```python
from build123d import *

# Parameters (mm, degrees)
SKETCH2_R          = 10.5
SKETCH2_R_2        = 8
CUT_EXTRUDE1_DEPTH = 1
CUT_EXTRUDE2_START = -1
SKETCH3_R          = 10.5
SKETCH3_R_2        = 8
CUT_EXTRUDE2_DEPTH = 1


with BuildPart() as part:
    # Sketch1 → Revolve1 (revolve)
    with BuildSketch(Plane.XY, mode=Mode.PRIVATE) as revolve1_sk:
        Polygon((0, 6), (6, 6), (6, 12), (1.5, 12), (1.5, 13.25), (0, 13.25), align=None)
    revolve(revolve1_sk.sketch.rotate(Axis((0, 0, 0), (1, 0, 0)), 90), axis=Axis((0, 0, 0), (1, 0, 0)))

    # Sketch2 → Cut-Extrude1 (cut)
    with BuildSketch(Plane(origin=(6, 0, 0), x_dir=(0, 0, -1), z_dir=(1, 0, 0))):
        Circle(SKETCH2_R)
        Circle(SKETCH2_R_2, mode=Mode.SUBTRACT)
    extrude(amount=-CUT_EXTRUDE1_DEPTH, mode=Mode.SUBTRACT)

    # Sketch3 → Cut-Extrude2 (cut)
    with BuildSketch(Plane.ZY.offset(CUT_EXTRUDE2_START)):
        with Locations(Location((0, 0, 0), (0, 0, 180))):
            Circle(SKETCH3_R)
        with Locations(Location((0, 0, 0), (0, 0, 180))):
            Circle(SKETCH3_R_2, mode=Mode.SUBTRACT)
    extrude(amount=CUT_EXTRUDE2_DEPTH, mode=Mode.SUBTRACT)


solid = part.part
```
Source: CAD feature listing. Evaluate the final solid. Frame: model axes, mm. A direction names the side the tool comes from. Round coordinates to 2 decimals unless told otherwise and drop trailing zeros. Write each loop counter-clockwise with the first axis right and the second up, starting at its lowest first coordinate (ties: lowest second). Pieces come first, ordered by that corner, then holes. Notation, with made-up numbers: M 52,-10 L 86,-10 A24 cw 86,5 Z; hole C -9,0 d5. An arc over 180 degrees is marked long. Use CSV: the item, a comma, the result in double quotes. Start each with the question number.
Q1. First-contact query: P1, Ø1, axis at x = 1, z = 1.5, coming from the +Y side; P2, Ø2, axis at x = 1, z = -9, coming from the +Y side; P3, Ø2, axis at x = 1, y = 4.5, coming from the -Z side. Flat tips, straight axial feed; report the tip coordinate or a pass-through.
Q2. Cut plane D-D on y = 11.5. Output: boundary loops of the cut face in (x, z).
Q3. Access query for faces 1 (the face through (5.51, -7.81, 1.73)), 2 (the face through (0.74, -13.137, -1.725)), 3 (the face through (0.51, 7.81, 1.73)). Directions: +Z, -Z, +X, -X, +Y, -Y. A direction counts if a zero-diameter tool reaches every point of the face in a straight line with its end or side. Return the directions, or none.
Q4. Line query: line 1 (Y direction, x = 5.3, z = 0); line 2 (Y direction, x = 1.9, z = 0); line 3 (Y direction, x = 0.55, z = -6.25). Output: solid intervals per line, ascending. Write a range as from..to.
Q5. Cut plane C-C on x = 0.5. Output: boundary loops of the cut face in (y, z), plus the area to 3 significant figures.
Q6. Cut plane A-A on z = 0. Output: boundary loops of the cut face in (x, y), plus the area to 4 significant figures.
Q7. Pull-direction query (Y, two-part tool) for faces 4 (the face through (0.5, -3.2, -10)), 5 (the face through (3.718, -3.604, 11.446)), 6 (the face through (5.5, 3.2, -10)), 7 (the face through (6, 11, 0)); classes: +Y half, -Y half, draft (parallel to the pull), parting line (faces both ways), or undercut.
Results found:
1,P1,"y = 13.21"
1,P2,"y = 10.56"
1,P3,"z = -12.78"
2,outline,"M 0,-6.58 L 1.5,-6.58 L 1.5,-3.43 L 6,-3.43 L 6,3.43 L 1.5,3.43 L 1.5,6.58 L 0,6.58 Z"
3,face 1,"+X"
3,face 2,"+X, -X"
3,face 3,"-X"
4,line 1,"-12..-10.5, -8..-6, 6..8, 10.5..12"
4,line 2,"-12..-6, 6..12"
4,line 3,"-11.68..-8.44, -4.99..4.99, 8.44..11.68"
5,outline,"C 0,0 d26.5; C 0,0 d16; hole C 0,0 d21; hole C 0,0 d12"
5,area,"293 mm^2"
6,outline,"M 0,-13.25 L 1.5,-13.25 L 1.5,-12 L 6,-12 L 6,-10.5 L 5,-10.5 L 5,-8 L 6,-8 L 6,-6 L 0,-6 L 0,-8 L 1,-8 L 1,-10.5 L 0,-10.5 Z; M 0,6 L 6,6 L 6,8 L 5,8 L 5,10.5 L 6,10.5 L 6,12 L 1.5,12 L 1.5,13.25 L 0,13.25 L 0,10.5 L 1,10.5 L 1,8 L 0,8 Z"
6,area,"65.75 mm^2"
7,face 4,"undercut"
7,face 5,"parting line"
7,face 6,"undercut"
7,face 7,"draft"
